from build123d import *

# Parameters (mm, degrees)
SKETCH1_W              = 31
SKETCH1_H              = 30
BOSS_EXTRUDE1_DEPTH    = 25
SKETCH2_W              = 3
SKETCH2_H              = 20
CUT_EXTRUDE1_DEPTH     = 51.498103381
SKETCH3_W              = 17.5
SKETCH3_H              = 15
BOSS_EXTRUDE2_DEPTH    = 30
CHAMFER1_SIZE          = 5
CHAMFER1_SIZE2         = 1.819851171
FILLET1_R              = 3
M10_TAPPED_HOLE1_D     = 8.5
M10_TAPPED_HOLE1_DEPTH = 24.5
M10_TAPPED_HOLE1_TIP   = 2.553657631


with BuildPart() as part:
    # Sketch1 → Boss-Extrude1 (new body)
    with BuildSketch(Plane.XY):
        with Locations((-16.516533934, 15.197368421)):
            Rectangle(SKETCH1_W, SKETCH1_H)
    extrude(amount=BOSS_EXTRUDE1_DEPTH)

    # Sketch2 → Cut-Extrude1 (cut, through all)
    with BuildSketch(Plane.XZ.offset(-0.197368421)):
        with Locations((-30.516533934, 15)):
            Rectangle(SKETCH2_W, SKETCH2_H)
        with Locations((-2.516533934, 15)):
            Rectangle(SKETCH2_W, SKETCH2_H)
    extrude(amount=-CUT_EXTRUDE1_DEPTH, mode=Mode.SUBTRACT)

    # Sketch3 → Boss-Extrude2 (add, through all)
    with BuildSketch(Plane(origin=(0, 30.197368421, 0), x_dir=(1, 0, 0), z_dir=(0, 1, 0))):
        with Locations((4.733466066, -17.5)):
            Rectangle(SKETCH3_W, SKETCH3_H)
        with Locations((-37.766533934, -17.5)):
            Rectangle(SKETCH3_W, SKETCH3_H)
    extrude(amount=-BOSS_EXTRUDE2_DEPTH)

    # Chamfer1
    chamfer1_edges = [part.edges().sort_by_distance(p)[0] for p in [
        (-16.516533934, 30.197368421, 25),
    ]]
    chamfer1_side = [part.faces().sort_by_distance(p)[0] for p in [
        (-16.516533934, 30.197368421, 14.470338983),
    ]]
    chamfer(chamfer1_edges, length=CHAMFER1_SIZE, length2=CHAMFER1_SIZE2, reference=chamfer1_side[0])

    # Fillet1
    fillet1_edges = [part.edges().sort_by_distance(p)[0] for p in [
        (-16.516533934, 28.37751725, 25),
        (-16.516533934, 30.197368421, 20),
    ]]
    fillet(fillet1_edges, radius=FILLET1_R)

    # M10 Tapped Hole1
    with Locations(Plane(origin=(0, 0.197368421, 0), x_dir=(-1, 0, 0), z_dir=(0, -1, 0))):
        with Locations((16.516533934, -10)):
            Hole(M10_TAPPED_HOLE1_D / 2, depth=M10_TAPPED_HOLE1_DEPTH)
            with Locations((0, 0, -(M10_TAPPED_HOLE1_DEPTH + M10_TAPPED_HOLE1_TIP / 2))):  # 118° drill point
                Cone(0, M10_TAPPED_HOLE1_D / 2, M10_TAPPED_HOLE1_TIP, mode=Mode.SUBTRACT)


solid = part.part
CAD build for the part. Positions are in the model's coordinates, mm. A direction names the side the tool comes from. Round coordinates to 2 decimals unless told otherwise and drop trailing zeros. Loops run counter-clockwise (first coordinate to the right, second up) from the corner with the lowest first, then second, coordinate; pieces in that order, holes last. Notation, with made-up numbers: M 56.5,-31.75 L 93.5,-31.75 A31 ccw 93.5,-5.75 Z; hole C 54,46 d2. An arc over 180 degrees is marked long. One line per question, with ' | ' between items. Start each with the question number.
Item 1: Two-plate mould, pull along X, no slides. Class faces 4 (the conical face through (-17.22, 26.81, 9.78)), 5 (the flat face through (-17, 0.197, 15)), 6 (the flat face through (-29.017, 15, 7)): pulls with the +X half, pulls with the -X half, needs draft (parallel to the pull), parting line crosses it, or undercut.
Item 2: Cut at D-D, the plane z = 4. Write the cut outline in (x, y).
Item 3: Pin check, flat tips, straight feed: pin 1 Ø12 at (x, z) = (-2.5, 9) entering from +Y; pin 2 Ø2.5 at (y, z) = (14, 7.5) entering from -X; pin 3 Ø2.5 at (y, z) = (16, 3) entering from +X; pin 4 Ø2.5 at (y, z) = (9.5, 2.5) entering from -X. Stop position of each tip, or through.
Item 4: Which spindle directions (+Z, -Z, +X, -X, +Y, -Y) get a long thin tool onto all of the face, cutting with end or side? Do faces 1 (the flat face through (-4.017, 15, 7)), 2 (the cylindrical face through (-19.889, 12.619, 12.586)), 3 (the flat face through (-32.017, 15, 2)). Say none if no direction does.
Item 5: Cut at B-B, the plane y = 20.5. Write the cut outline in (x, z), plus the area to 3 significant figures.
Item 6: Cut at A-A, the plane x = -2. Write the cut outline in (y, z), plus the area to 3 significant figures.
Item 7: Cut at C-C, the plane x = -33. Write the cut outline in (y, z).
Item 8: Wall check: line 1 (Z direction, x = -31, y = 13.25); line 2 (X direction, y = 7.75, z = 1.75); line 3 (Z direction, x = -41.5, y = 3.5). Give the ranges that are in metal, low to high.
Responses:
1) face 4: undercut | face 5: needs draft | face 6: pulls with the -X half
2) outline: M -32.02,0.2 L -1.02,0.2 L -1.02,30.2 L -32.02,30.2 Z
3) pin 1: stops at y = 30.2 | pin 2: stops at x = -29.02 | pin 3: stops at x = -1.02 | pin 4: stops at x = -32.02
4) face 1: +X, +Y, -Y | face 2: -Y | face 3: -Z, -X, +Y, -Y
5) outline: M -46.52,10 L -29.02,10 L -29.02,5 L -32.02,5 L -32.02,0 L -1.02,0 L -1.02,5 L -4.02,5 L -4.02,10 L 13.48,10 L 13.48,25 L -46.52,25 Z; hole C -16.52,10 d8.5 | area: 1,120 mm²
6) outline: M 0.2,0 L 30.2,0 L 30.2,5 L 0.2,5 Z; M 0.2,10 L 30.2,10 L 30.2,19.47 A3 ccw 30.02,20.5 L 29.1,23.03 A3 ccw 26.28,25 L 0.2,25 Z | area: 595 mm²
7) outline: M 0.2,10 L 30.2,10 L 30.2,19.47 A3 ccw 30.02,20.5 L 29.1,23.03 A3 ccw 26.28,25 L 0.2,25 Z
8) line 1: z = 0 to 5, 10 to 25 | line 2: x = -32.02 to -1.02 | line 3: z = 10 to 25
